Model file for the job. Use its own axes, mm. Face numbers are marked on the shaded views. A direction names the side the tool comes from. Give positions to 0.01 mm unless a question says otherwise; leave off trailing zeros. Order: outer loops, then holes, each group sorted by start corner. A loop starts at its lowest first (then second) coordinate and runs counter-clockwise, first axis right, second up. Notation, with made-up numbers: M -32,37.5 L -16,37.5 A16 ccw -16,47.5 Z; hole C 27,71.5 d2. An arc over 180 degrees is marked long. Return JSON: item names as keys, results as strings. Group by question number.
1. Wall check: probe 1 along Y at (x, z) = (-60.5, 25); probe 2 along Y at (x, z) = (-38.5, 50); probe 3 along Z at (x, y) = (33.5, -199). Give the ranges that are in metal, low to high. Write a range as [from, to].
2. Pin check, flat tips, straight feed: pin 1 (5 mm diameter, centred on x = -63, y = -37.5, fed in from +Z); pin 2 (12 mm diameter, centred on y = -36.5, z = 27, fed in from -X); pin 3 (12 mm diameter, centred on y = 223, z = 26, fed in from -X). Stop position of each tip, or through.
3. Slice it at C-C on x = 53.5. List the corners of the cut face in (y, z).
4. Slice it at A-A on x = -200. List the corners of the cut face in (y, z).
5. 3-axis set-ups, long thin cutter, end or side, ignore diameter. For the marked faces 1 and 2: which of +Z, -Z, +X, -X, +Y, -Y reach the whole face in a straight line?
6. Slice it at D-D on x = 0. List the corners of the cut face in (y, z).
7. Slice it at B-B on y = 0. List the corners of the cut face in (x, z).
8. Two-plate mould, pull along X, no slides. Class the marked faces 3 and 4: released by +X, released by -X, zero draft, split by the parting line, or undercut.
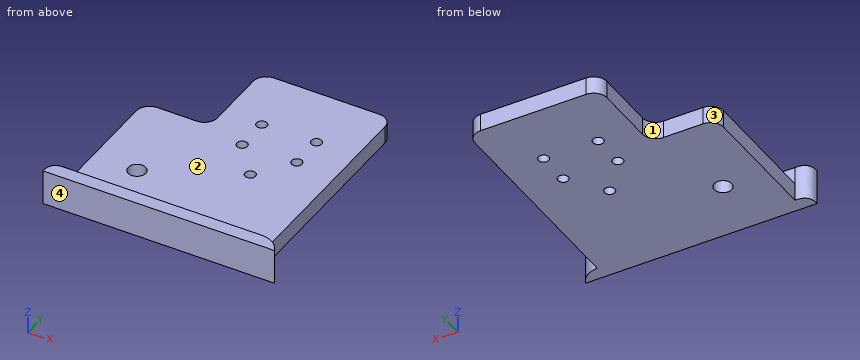
from build123d import *

# Parameters (mm, degrees)
SKETCH1_W           = 600
SKETCH1_H           = 600
BOSS_EXTRUDE1_DEPTH = 40
SKETCH2_R           = 20
CUT_EXTRUDE1_DEPTH  = 40
SKETCH3_R           = 12
CUT_EXTRUDE2_DEPTH  = 60
SKETCH4_R           = 12
CUT_EXTRUDE3_DEPTH  = 90
SKETCH5_W           = 150
SKETCH5_H           = 600
CUT_EXTRUDE4_DEPTH  = 100
SKETCH6_W           = 150
SKETCH6_H           = 200
CUT_EXTRUDE5_DEPTH  = 100
SKETCH7_W           = 450
SKETCH7_H           = 90
CUT_EXTRUDE6_DEPTH  = 100
SKETCH9_R           = 12
CUT_EXTRUDE7_DEPTH  = 50
FILLET1_R           = 30
BOSS_EXTRUDE2_DEPTH = 80


with BuildPart() as part:
    # Sketch1 → Boss-Extrude1 (new body)
    with BuildSketch(Plane.XY):
        Rectangle(SKETCH1_W, SKETCH1_H)
    extrude(amount=BOSS_EXTRUDE1_DEPTH)

    # Sketch2 → Cut-Extrude1 (cut)
    with BuildSketch(Plane.XY.offset(40)):
        with Locations((-200, -100)):
            Circle(SKETCH2_R)
    extrude(amount=-CUT_EXTRUDE1_DEPTH, mode=Mode.SUBTRACT)

    # Sketch3 → Cut-Extrude2 (cut)
    with BuildSketch(Plane.XY.offset(40)):
        Circle(SKETCH3_R)
    extrude(amount=-CUT_EXTRUDE2_DEPTH, mode=Mode.SUBTRACT)

    # Sketch4 → Cut-Extrude3 (cut)
    with BuildSketch(Plane.XY.offset(40)):
        with Locations((-63.335275248, 77.386322495)):
            Circle(SKETCH4_R)
        with Locations((59.168411159, 80.616990275)):
            Circle(SKETCH4_R)
    extrude(amount=-CUT_EXTRUDE3_DEPTH, mode=Mode.SUBTRACT)

    # Sketch5 → Cut-Extrude4 (cut)
    with BuildSketch(Plane.XY.offset(40)):
        with Locations((225, 0)):
            Rectangle(SKETCH5_W, SKETCH5_H)
    extrude(amount=-CUT_EXTRUDE4_DEPTH, mode=Mode.SUBTRACT)

    # Sketch6 → Cut-Extrude5 (cut)
    with BuildSketch(Plane.XY.offset(40)):
        with Locations((-225, 200)):
            Rectangle(SKETCH6_W, SKETCH6_H)
    extrude(amount=-CUT_EXTRUDE5_DEPTH, mode=Mode.SUBTRACT)

    # Sketch7 → Cut-Extrude6 (cut)
    with BuildSketch(Plane.XY.offset(40)):
        with Locations((-75, -255)):
            Rectangle(SKETCH7_W, SKETCH7_H)
    extrude(amount=-CUT_EXTRUDE6_DEPTH, mode=Mode.SUBTRACT)

    # Sketch9 → Cut-Extrude7 (cut)
    with BuildSketch(Plane.XY.offset(40)):
        with Locations((-63.335275248, 154.386322495)):
            Circle(SKETCH9_R)
        with Locations((59.168411159, 157.616990275)):
            Circle(SKETCH9_R)
    extrude(amount=-CUT_EXTRUDE7_DEPTH, mode=Mode.SUBTRACT)

    # Fillet1
    fillet1_edges = [part.edges().sort_by_distance(p)[0] for p in [
        (150, 300, 20),
        (-300, 100, 20),
        (-150, 300, 20),
        (-150, 100, 20),
    ]]
    fillet(fillet1_edges, radius=FILLET1_R)

    # Sketch10 → Boss-Extrude2 (add)
    with BuildSketch(Plane(origin=(0, 0, 0), x_dir=(-1, 0, 0), z_dir=(0, 0, -1))):
        with BuildLine():
            Line((-150, -210), (300, -210))
            add(Edge.make_bspline(
                [(300, -210), (333.145645994, -208.556298113), (332.053728057, -241.264865933)],
                knots=[0, 0, 0, 1, 1, 1], degree=2))
            Line((332.053728057, -241.264865933), (-194.702453995, -241.264865933))
            add(Edge.make_bspline(
                [(-150, -210), (-181.312836573, -212.059215881), (-194.702453995, -241.264865933)],
                knots=[0, 0, 0, 1, 1, 1], degree=2))
        make_face()
    extrude(amount=-BOSS_EXTRUDE2_DEPTH)


solid = part.part
Result:
{
 "1": {"probe 1": "y = [-241.26, 65.73], [89.05, 142.73], [166.05, 300]", "probe 2": "y = [-241.26, -210]", "probe 3": "z = [0, 40]"},
 "2": {"pin 1": "stops at z = 40", "pin 2": "stops at x = -300", "pin 3": "stops at x = -150"},
 "3": {"outline": "M -241.26,0 L 70.04,0 L 70.04,40 L -210,40 L -210,80 L -241.26,80 Z; M 91.19,0 L 147.04,0 L 147.04,40 L 91.19,40 Z; M 168.19,0 L 300,0 L 300,40 L 168.19,40 Z"},
 "4": {"outline": "M -241.26,0 L -120,0 L -120,40 L -210,40 L -210,80 L -241.26,80 Z; M -80,0 L 100,0 L 100,40 L -80,40 Z"},
 "5": {"face 1": "+Z, -Z, -X, +Y", "face 2": "+Z, +X, -X, +Y"},
 "6": {"outline": "M -241.26,0 L -12,0 L -12,40 L -210,40 L -210,80 L -241.26,80 Z; M 12,0 L 300,0 L 300,40 L 12,40 Z"},
 "7": {"outline": "M -300,0 L -12,0 L -12,40 L -300,40 Z; M 12,0 L 150,0 L 150,40 L 12,40 Z"},
 "8": {"face 3": "released by -X", "face 4": "zero draft"}
}
